Work out the finished part from the listing and answer in its coordinate system (mm). A direction names the side the tool comes from. Give positions to 0.01 mm unless a question says otherwise; leave off trailing zeros. Write each loop counter-clockwise with the first axis right and the second up, starting at its lowest first coordinate (ties: lowest second). Pieces come first, ordered by that corner, then holes.
1) A tool of negligible diameter and unlimited length cuts with its end or side. For faces 4 (the face through (-20, -1, 3)), 5 (the face through (16, -1, 3)), from which of +Z, -Z, +X, -X, +Y, -Y can it reach the whole face along a straight path? Write none if from no direction.
2) Determine the mould class of faces 1 (the face through (-16.4, 3.1, -180)), 2 (the face through (0, 40, 3)), 3 (the face through (0, -36, 3)) for opening direction Y: pulls with the +Y half, pulls with the -Y half, needs draft (parallel to the pull), parting line crosses it, or undercut.
3) Find section C-C (z = -63). Determine the outline of the cut face in (x, y).
4) Straight lines are drawn through the part: probe 1 along Y at (x, z) = (8.5, 92); probe 2 along X at (y, z) = (7.5, -107). For each, find the intervals that lie inside material, in ascending order.
5) Find section B-B (x = 1). Determine the outline of the cut face in (y, z), plus the area to 3 significant figures.
6) Find section A-A (y = 0.5). Determine the outline of the cut face in (x, z).
```python
from build123d import *

# Parameters (mm, degrees)
SKETCH_1_W      = 40
SKETCH_1_H      = 80
SKETCH_1_W_2    = 32
SKETCH_1_H_2    = 72
EXTRUDE_1_DEPTH = 180


with BuildPart() as part:
    # 草图1 → 凸台-拉伸1 (new, symmetric)
    with BuildSketch(Plane.XY):
        Rectangle(SKETCH_1_W, SKETCH_1_H)
        Rectangle(SKETCH_1_W_2, SKETCH_1_H_2, mode=Mode.SUBTRACT)
    extrude(amount=EXTRUDE_1_DEPTH, both=True)


solid = part.part
```
Results:
1. face 4: +Z, -Z, -X, +Y, -Y
1. face 5: +Z, -Z
2. face 1: needs draft
2. face 2: pulls with the +Y half
2. face 3: undercut
3. outline: (-20, -40) - (20, -40) - (20, 40) - (-20, 40) - close; hole (-16, -36) - (16, -36) - (16, 36) - (-16, 36) - close
4. probe 1: y = -40 to -36, 36 to 40
4. probe 2: x = -20 to -16, 16 to 20
5. outline: (-40, -180) - (-36, -180) - (-36, 180) - (-40, 180) - close; (36, -180) - (40, -180) - (40, 180) - (36, 180) - close
5. area: 2,880 mm2
6. outline: (-20, -180) - (-16, -180) - (-16, 180) - (-20, 180) - close; (16, -180) - (20, -180) - (20, 180) - (16, 180) - close
